```python
from build123d import *

# Parameters (mm, degrees)
BOSS_EXTRUDE1_DEPTH = 70


with BuildPart() as part:
    # Sketch1 → Boss-Extrude1 (new body)
    with BuildSketch(Plane.XY):
        Polygon((4, -4), (4, -56), (-4, -56), (-4, -4), (-50, -4), (-50, 4), (-4, 4), (-4, 94), (4, 94), (4, 4), (50, 4), (50, -4), align=None)
    extrude(amount=BOSS_EXTRUDE1_DEPTH)


solid = part.part
```
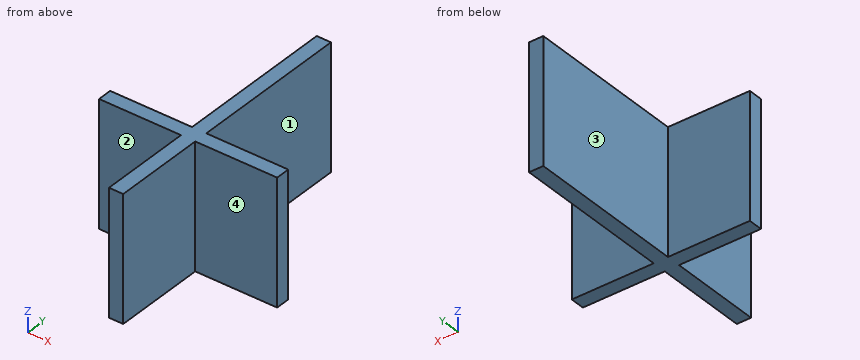
Geometry check sheet. Reference: the model listing, model coordinates, mm. Face numbers are marked on the shaded views. A direction names the side the tool comes from. Coordinates: 2 decimals unless noted, no trailing zeros. Loops run counter-clockwise (first coordinate to the right, second up) from the corner with the lowest first, then second, coordinate; pieces in that order, holes last.
Item 1: Sectioned sample at A-A, the plane z = 28. Record the boundary of the cut face in (x, y), then the cut area to 3 significant figures.
Item 2: Access from +Z, -Z, +X, -X, +Y, -Y to the whole of each face (thin tool, end or side, straight path). Record for the marked faces 1, 2, 3 and 4.
Item 3: Sectioned sample at B-B, the plane x = -13. Record the boundary of the cut face in (y, z), then the cut area to 3 significant figures.
Item 4: Go/stop test with flat-tipped pins: pin 1 Ø3 at (y, z) = (-28.5, 18) entering from +X; pin 2 Ø5 at (x, z) = (-13, 8) entering from +Y; pin 3 Ø3 at (x, z) = (23.5, 28.5) entering from -Y. Record where each tip stops, or that it passes through.
Item 5: Thickness scan on line 1 (Y direction, x = 39, z = 16). Record the ranges inside material, lowest first.
Check result:
1. outline: (-50, -4) - (-4, -4) - (-4, -56) - (4, -56) - (4, -4) - (50, -4) - (50, 4) - (4, 4) - (4, 94) - (-4, 94) - (-4, 4) - (-50, 4) - close
1. area: 1,940 mm2
2. face 1: +Z, -Z, +X, +Y
2. face 2: +Z, -Z, -X, -Y
2. face 3: +Z, -Z, -X, +Y
2. face 4: +Z, -Z, +X, -Y
3. outline: (-4, 0) - (4, 0) - (4, 70) - (-4, 70) - close
3. area: 560 mm2
4. pin 1: stops at x = 4
4. pin 2: stops at y = 4
4. pin 3: stops at y = -4
5. line 1: y = -4 to 4
